```python
from build123d import *

# Parameters (mm, degrees)
SKETCH_1_W          = 40.33
SKETCH_1_H          = 28.16
EXTRUDE_1_DEPTH     = 11.1
SKETCH_2_W          = 12
SKETCH_2_H          = 2.45
CUT_EXTRUDE_1_DEPTH = 10
SKETCH_3_W          = 0.5
SKETCH_3_H          = 0.5
EXTRUDE_2_DEPTH     = 9
SKETCH_4_W          = 0.5
SKETCH_4_H          = 0.5
EXTRUDE_3_DEPTH     = 9
SKETCH_5_W          = 0.5
SKETCH_5_H          = 0.5
EXTRUDE_4_DEPTH     = 9
SKETCH_6_W          = 0.5
SKETCH_6_H          = 0.5
EXTRUDE_5_DEPTH     = 9
SKETCH_7_W          = 6.06
SKETCH_7_H          = 6.06
EXTRUDE_6_DEPTH     = 4
SKETCH_8_W          = 6.06
SKETCH_8_H          = 6.06
EXTRUDE_7_DEPTH     = 4
CHAMFER_1_SIZE      = 0.35
FILLET_1_R          = 1
FILLET_2_R          = 2


with BuildPart() as part:
    # 草图1 → 凸台-拉伸1 (new body)
    with BuildSketch(Plane(origin=(0, 11.1, 0), x_dir=(1, 0, 0), z_dir=(0, 1, 0))):
        Rectangle(SKETCH_1_W, SKETCH_1_H)
    extrude(amount=-EXTRUDE_1_DEPTH)

    # 草图2 → 切除-拉伸1 (cut)
    with BuildSketch(Plane.XY.offset(14.08)):
        with Locations((-5.865, 6.775)):
            Rectangle(SKETCH_2_W, SKETCH_2_H)
    extrude(amount=-CUT_EXTRUDE_1_DEPTH, mode=Mode.SUBTRACT)

    # 草图3 → 凸台-拉伸2 (add)
    with BuildSketch(Plane.XY.offset(4.08)):
        with Locations((-4.715, 6.775)):
            Rectangle(SKETCH_3_W, SKETCH_3_H)
    extrude(amount=EXTRUDE_2_DEPTH)

    # 草图4 → 凸台-拉伸3 (add)
    with BuildSketch(Plane.XY.offset(4.08)):
        with Locations((-9.315, 6.775)):
            Rectangle(SKETCH_4_W, SKETCH_4_H)
    extrude(amount=EXTRUDE_3_DEPTH)

    # 草图5 → 凸台-拉伸4 (add)
    with BuildSketch(Plane.XY.offset(4.08)):
        with Locations((-7.015, 6.775)):
            Rectangle(SKETCH_5_W, SKETCH_5_H)
    extrude(amount=EXTRUDE_4_DEPTH)

    # 草图6 → 凸台-拉伸5 (add)
    with BuildSketch(Plane.XY.offset(4.08)):
        with Locations((-2.415, 6.775)):
            Rectangle(SKETCH_6_W, SKETCH_6_H)
    extrude(amount=EXTRUDE_5_DEPTH)

    # 草图7 → 凸台-拉伸6 (add)
    with BuildSketch(Plane.ZY.offset(20.165)):
        with Locations((0, 5.55)):
            Rectangle(SKETCH_7_W, SKETCH_7_H)
    extrude(amount=EXTRUDE_6_DEPTH)

    # 草图8 → 凸台-拉伸7 (add)
    with BuildSketch(Plane(origin=(20.165, 0, 0), x_dir=(0, 0, -1), z_dir=(1, 0, 0))):
        with Locations((0, 5.55)):
            Rectangle(SKETCH_8_W, SKETCH_8_H)
    extrude(amount=EXTRUDE_7_DEPTH)

    # 倒角1
    chamfer_1_edges = [part.edges().sort_by_distance(p)[0] for p in [
        (-11.865, 8, 9.08),
        (0.135, 8, 9.08),
    ]]
    chamfer(chamfer_1_edges, length=CHAMFER_1_SIZE)

    # 圆角1
    fillet_1_edges = [part.edges().sort_by_distance(p)[0] for p in [
        (-22.165, 2.52, -3.03),
        (-22.165, 2.52, 3.03),
        (-22.165, 8.58, 3.03),
        (-22.165, 8.58, -3.03),
        (22.165, 2.52, 3.03),
        (22.165, 2.52, -3.03),
        (22.165, 8.58, -3.03),
        (22.165, 8.58, 3.03),
    ]]
    fillet(fillet_1_edges, radius=FILLET_1_R)

    # 圆角2
    fillet_2_edges = [part.edges().sort_by_distance(p)[0] for p in [
        (20.165, 5.55, -14.08),
        (20.165, 5.55, 14.08),
        (-20.165, 5.55, 14.08),
        (-20.165, 5.55, -14.08),
    ]]
    fillet(fillet_2_edges, radius=FILLET_2_R)


solid = part.part
```
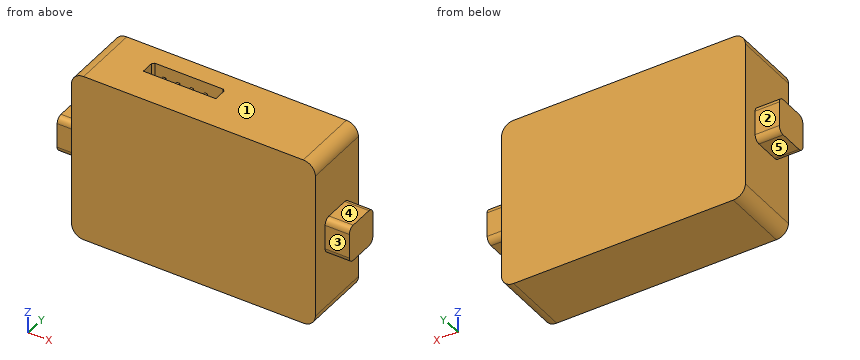
Read the model definition and answer for the solid it produces. Units are mm, in the model's axes. Face numbers are marked on the shaded views. A direction names the side the tool comes from. Round coordinates to 2 decimals unless told otherwise and drop trailing zeros. Write each loop counter-clockwise with the first axis right and the second up, starting at its lowest first coordinate (ties: lowest second). Pieces come first, ordered by that corner, then holes. Notation, with made-up numbers: (41.25, 37) - (75.25, 37) arc R13 ccw to (75.25, 55) - close; hole circle Ø10 at (-5, 20). An arc over 180 degrees is marked (long way). One line per item, written item: value.
Q1. Find section D-D (x = 19.5). Determine the outline of the cut face in (y, z), and give its area (3 significant figures).
The answers:
outline: (0, -13.57) - (11.1, -13.57) - (11.1, 13.57) - (0, 13.57) - close
area: 301 mm2
Q2. Which of the six approach directions +Z, -Z, +X, -X, +Y, -Y give full straight-line access (tool end or side, diameter ignored) to the marked faces 1, 2, 3, 4 and 5?
The answers:
face 1: +Z, +X, -X, +Y, -Y
face 2: +Z, -Z, -X, +Y
face 3: +Z, -Z, +X, -Y
face 4: +Z, +X, +Y, -Y
face 5: -Z, -X, +Y, -Y
Q3. Each of these flat-tipped pins is pushed along its axis until it touches: P1, Ø3, axis at x = 22.5, y = 6, coming from the +Z side; P2, Ø2, axis at y = 6.5, z = -10.5, coming from the +X side (3 decimals); P3, Ø4.5, axis at x = -21.5, y = 5, coming from the -Z side. Where does it stop, or does it pass through?
The answers:
P1: stops at z = 3.03
P2: stops at x = 20.165
P3: stops at z = -13.76
Q4. Find section B-B (y = 9.5). Determine the outline of the cut face in (x, z) (3 decimals), and give its area (3 significant figures).
The answers:
outline: (-20.165, -12.08) arc R2 ccw to (-18.165, -14.08) - (18.165, -14.08) arc R2 ccw to (20.165, -12.08) - (20.165, 12.08) arc R2 ccw to (18.165, 14.08) - (-18.165, 14.08) arc R2 ccw to (-20.165, 12.08) - close
area: 1,130 mm2
Q5. Find section C-C (z = 0.5). Determine the outline of the cut face in (x, y) (3 decimals), and give its area (3 significant figures).
The answers:
outline: (-24.165, 2.52) - (-20.165, 2.52) - (-20.165, 0) - (20.165, 0) - (20.165, 2.52) - (24.165, 2.52) - (24.165, 8.58) - (20.165, 8.58) - (20.165, 11.1) - (-20.165, 11.1) - (-20.165, 8.58) - (-24.165, 8.58) - close
area: 496 mm2
Q6. Straight lines are drawn through the part: line 1 (X direction, y = 6.75, z = 4.75) (3 decimals); line 2 (Y direction, x = -8, z = 11); line 3 (X direction, y = 4.25, z = 10.5) (3 decimals). For each, find the intervals that lie inside material, in ascending order. Write a range as from..to.
The answers:
line 1: x = -20.165..-11.865, -9.565..-9.065, -7.265..-6.765, -4.965..-4.465, -2.665..-2.165, 0.135..20.165
line 2: y = 0..5.55, 8..11.1
line 3: x = -20.165..20.165
Q7. Find section A-A (z = 6.5). Determine the outline of the cut face in (x, y) (3 decimals), and give its area (3 significant figures).
The answers:
outline: (-20.165, 0) - (20.165, 0) - (20.165, 11.1) - (-20.165, 11.1) - close; (-9.565, 6.525) - (-9.065, 6.525) - (-9.065, 7.025) - (-9.565, 7.025) - close; (-7.265, 6.525) - (-6.765, 6.525) - (-6.765, 7.025) - (-7.265, 7.025) - close; (-4.965, 6.525) - (-4.465, 6.525) - (-4.465, 7.025) - (-4.965, 7.025) - close; (-2.665, 6.525) - (-2.165, 6.525) - (-2.165, 7.025) - (-2.665, 7.025) - close; hole (-11.865, 5.55) - (0.135, 5.55) - (0.135, 7.65) - (-0.215, 8) - (-11.515, 8) - (-11.865, 7.65) - close
area: 419 mm2
